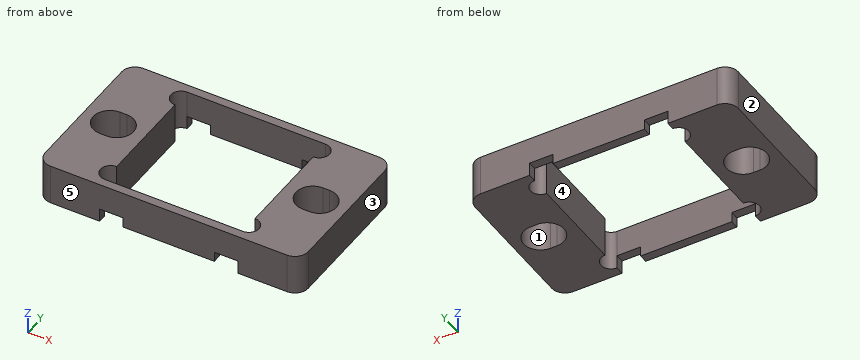
from build123d import *

# Parameters (mm, degrees)
SKETCH1_W           = 39
SKETCH1_H           = 23
SKETCH1_W_2         = 20.5
SKETCH1_H_2         = 20.5
BOSS_EXTRUDE1_DEPTH = 6
CUT_EXTRUDE1_REACH  = 32.745
SKETCH2_W           = 20.5
SKETCH2_H           = 4.35
SKETCH3_W           = 20.5
SKETCH3_H           = 1.25
BOSS_EXTRUDE2_DEPTH = 4.35
CUT_EXTRUDE2_REACH  = 32.745
CUT_EXTRUDE3_START  = -6
CUT_EXTRUDE3_DEPTH  = 6
CUT_EXTRUDE4_DEPTH  = 10
FILLET1_R           = 2


with BuildPart() as part:
    # Sketch1 → Boss-Extrude1 (new body)
    with BuildSketch(Plane.XY):
        Rectangle(SKETCH1_W, SKETCH1_H)
        Rectangle(SKETCH1_W_2, SKETCH1_H_2, mode=Mode.SUBTRACT)
    extrude(amount=BOSS_EXTRUDE1_DEPTH)

    # Cut-Extrude1: up to this face of the body (flat: up to its plane)
    cut_extrude1_end = Plane(part.part.faces().sort_by_distance((0, 11.5, 3))[0])
    # Sketch2 → Cut-Extrude1 (cut, up to the picked face)
    with BuildSketch(Plane.XZ.offset(11.5), mode=Mode.PRIVATE) as cut_extrude1_sk1:
        with Locations((0, 3.825)):
            Rectangle(SKETCH2_W, SKETCH2_H)
    cut_extrude1_tool1 = split(extrude(cut_extrude1_sk1.sketch, amount=-CUT_EXTRUDE1_REACH, mode=Mode.PRIVATE), bisect_by=cut_extrude1_end, keep=Keep.BOTH, mode=Mode.PRIVATE)
    add(cut_extrude1_tool1.solids().sort_by(Axis((0, -11.5, 3.825), (0, 1, 0)))[0], mode=Mode.SUBTRACT)

    # Sketch3 → Boss-Extrude2 (add)
    with BuildSketch(Plane.XY.offset(6)):
        with Locations((0, 10.875)):
            Rectangle(SKETCH3_W, SKETCH3_H)
        with Locations((0, -10.875)):
            Rectangle(SKETCH3_W, SKETCH3_H)
    extrude(amount=-BOSS_EXTRUDE2_DEPTH)

    # Cut-Extrude2: up to this face of the body (flat: up to its plane)
    cut_extrude2_end = Plane(part.part.faces().sort_by_distance((0, 11.5, 3))[0])
    # Sketch4 → Cut-Extrude2 (cut, up to the picked face)
    with BuildSketch(Plane.XZ.offset(11.5), mode=Mode.PRIVATE) as cut_extrude2_sk1:
        Polygon((6.75, 0.5), (6.75, 2), (10.25, 2), (10.25, 0), (6.75, 0), (-6.75, 0), (-10.25, 0), (-10.25, 2), (-6.75, 2), (-6.75, 0.5), align=None)
    cut_extrude2_tool1 = split(extrude(cut_extrude2_sk1.sketch, amount=-CUT_EXTRUDE2_REACH, mode=Mode.PRIVATE), bisect_by=cut_extrude2_end, keep=Keep.BOTH, mode=Mode.PRIVATE)
    add(cut_extrude2_tool1.solids().sort_by(Axis((6.955973, -11.5, 1.25), (0, 1, 0)))[0], mode=Mode.SUBTRACT)

    # Sketch5 → Cut-Extrude3 (cut)
    with BuildSketch(Plane(origin=(0, 0, 0), x_dir=(-1, 0, 0), z_dir=(0, 0, -1)).offset(CUT_EXTRUDE3_START)):
        with BuildLine():
            Line((-10.25, 10.25), (10.25, 10.25))
            ThreePointArc((10.25, 10.25), (11.75, 8.75), (10.25, 7.25))
            Line((10.25, 7.25), (-10.25, 7.25))
            ThreePointArc((-10.25, 7.25), (-11.75, 8.75), (-10.25, 10.25))
        make_face()
        with BuildLine():
            Line((-10.25, -7.25), (10.25, -7.25))
            ThreePointArc((10.25, -7.25), (11.75, -8.75), (10.25, -10.25))
            Line((10.25, -10.25), (-10.25, -10.25))
            ThreePointArc((-10.25, -10.25), (-11.75, -8.75), (-10.25, -7.25))
        make_face()
    extrude(amount=CUT_EXTRUDE3_DEPTH, mode=Mode.SUBTRACT)

    # Sketch6 → Cut-Extrude4 (cut)
    with BuildSketch(Plane.XY.offset(6)):
        with BuildLine():
            Line((-15.5, 2.4), (-14.5, 2.4))
            ThreePointArc((-14.5, 2.4), (-12, -0.1), (-14.5, -2.6))
            Line((-14.5, -2.6), (-15.5, -2.6))
            ThreePointArc((-15.5, -2.6), (-18, -0.1), (-15.5, 2.4))
        make_face()
        with BuildLine():
            Line((14.5, 2.5), (15.5, 2.5))
            ThreePointArc((15.5, 2.5), (18, 0), (15.5, -2.5))
            Line((15.5, -2.5), (14.5, -2.5))
            ThreePointArc((14.5, -2.5), (12, 0), (14.5, 2.5))
        make_face()
    extrude(amount=-CUT_EXTRUDE4_DEPTH, mode=Mode.SUBTRACT)

    # Fillet1
    fillet1_edges = [part.edges().sort_by_distance(p)[0] for p in [
        (19.5, -11.5, 3),
        (-19.5, -11.5, 3),
        (-19.5, 11.5, 3),
        (19.5, 11.5, 3),
    ]]
    fillet(fillet1_edges, radius=FILLET1_R)


solid = part.part
Input: part model. Units: mm. Frame: model coordinates. Face numbers are marked on the shaded views. A direction names the side the tool comes from. Round coordinates to 2 decimals unless told otherwise and drop trailing zeros. Order: outer loops, then holes, each group sorted by start corner. A loop starts at its lowest first (then second) coordinate and runs counter-clockwise, first axis right, second up.
1. Set-up query: the marked faces 4 and 5. Return all of +Z, -Z, +X, -X, +Y, -Y with unobstructed straight access to the full face (end or side cutting, diameter ignored); none if empty.
The answers:
face 4: +Z, -Z
face 5: +Z, -Z, +X, -X, -Y
2. Cut plane A-A, the plane y = -5.5. Output: boundary loops of the cut face in (x, z).
The answers:
outline: (-19.5, 0) - (-10.25, 0) - (-10.25, 6) - (-19.5, 6) - close; (10.25, 0) - (19.5, 0) - (19.5, 6) - (10.25, 6) - close
3. Cut plane C-C, the plane z = 4.35. Output: boundary loops of the cut face in (x, y).
The answers:
outline: (-19.5, -9.5) arc R2 ccw to (-17.5, -11.5) - (17.5, -11.5) arc R2 ccw to (19.5, -9.5) - (19.5, 9.5) arc R2 ccw to (17.5, 11.5) - (-17.5, 11.5) arc R2 ccw to (-19.5, 9.5) - close; hole (-15.5, -2.6) - (-14.5, -2.6) arc R2.5 ccw to (-14.5, 2.4) - (-15.5, 2.4) arc R2.5 ccw to start; hole (-10.25, -10.25) - (10.25, -10.25) arc R1.5 ccw to (10.25, -7.25) - (10.25, 7.25) arc R1.5 ccw to (10.25, 10.25) - (-10.25, 10.25) arc R1.5 ccw to (-10.25, 7.25) - (-10.25, -7.25) arc R1.5 ccw to start; hole (14.5, -2.5) - (15.5, -2.5) arc R2.5 ccw to (15.5, 2.5) - (14.5, 2.5) arc R2.5 ccw to start
4. Material intervals for line 1 (X direction, y = 0, z = 2.15); line 2 (Y direction, x = -0.5, z = 4.7); line 3 (X direction, y = 4, z = 1.3), sorted ascending.
The answers:
line 1: x = -19.5 to -18, -12 to -10.25, 10.25 to 12, 18 to 19.5
line 2: y = -11.5 to -10.25, 10.25 to 11.5
line 3: x = -19.5 to -10.25, 10.25 to 19.5
5. Pin query (flat end, axial travel): P1, Ø1.4, axis at y = -11, z = 1.5, coming from the +X side; P2, Ø1, axis at x = -8.5, y = 11, coming from the -Z side; P3, Ø1.4, axis at y = 11, z = 1, coming from the -X side; P4, Ø10, axis at x = -2.5, y = 1.5, coming from the +Z side. Return the tip coordinate at first contact, or that it passes through.
The answers:
P1: stops at x = 19.33
P2: stops at z = 2
P3: stops at x = -19.33
P4: passes through
6. Cut plane B-B, the plane x = 9. Output: boundary loops of the cut face in (y, z), then the cut area to 3 significant figures.
The answers:
outline: (-11.5, 2) - (-10.25, 2) - (-10.25, 6) - (-11.5, 6) - close; (10.25, 2) - (11.5, 2) - (11.5, 6) - (10.25, 6) - close
area: 10.0 mm2
7. Cut plane D-D, the plane y = 0. Output: boundary loops of the cut face in (x, z).
The answers:
outline: (-19.5, 0) - (-18, 0) - (-18, 6) - (-19.5, 6) - close; (-12, 0) - (-10.25, 0) - (-10.25, 6) - (-12, 6) - close; (10.25, 0) - (12, 0) - (12, 6) - (10.25, 6) - close; (18, 0) - (19.5, 0) - (19.5, 6) - (18, 6) - close
8. Mould query, pull axis X, two halves, no side actions, for the marked faces 1, 2 and 3. Classes: released by +X, released by -X, zero draft, split by the parting line, or undercut.
The answers:
face 1: undercut
face 2: released by -X
face 3: released by +X
